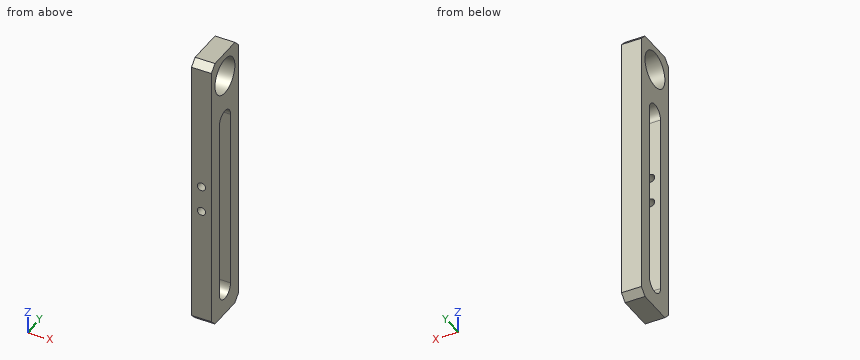
```python
from build123d import *

# Parameters (mm, degrees)
SKETCH1_W              = 85
SKETCH1_H              = 15
EXTRUDE1_DEPTH         = 6
M12X1_0_TAPPED_HOLE1_D = 11
CHAMFER1_SIZE          = 2
M3_TAPPED_HOLE1_D      = 2.5
M3_TAPPED_HOLE1_DEPTH  = 8.5
M3_TAPPED_HOLE1_TIP    = 0.751075774


with BuildPart() as part:
    # Sketch1 → Extrude1 (new body)
    with BuildSketch(Plane(origin=(0, 0, 0), x_dir=(0, 0, -1), z_dir=(1, 0, 0))):
        with Locations((42.5, -7.5)):
            Rectangle(SKETCH1_W, SKETCH1_H)
        with BuildLine():
            Line((22, -4.4), (77, -4.4))
            ThreePointArc((77, -4.4), (80.1, -7.5), (77, -10.6))
            Line((77, -10.6), (22, -10.6))
            ThreePointArc((22, -10.6), (18.9, -7.5), (22, -4.4))
        make_face(mode=Mode.SUBTRACT)
    extrude(amount=EXTRUDE1_DEPTH)

    # M12x1.0 Tapped Hole1 (through all)
    with Locations(Plane(origin=(6, 0, 0), x_dir=(0, 0, -1), z_dir=(1, 0, 0))):
        with Locations((7.5, -7.5)):
            Hole(M12X1_0_TAPPED_HOLE1_D / 2)

    # Chamfer1
    chamfer1_edges = [part.edges().sort_by_distance(p)[0] for p in [
        (3, 0, 0),
        (3, 0, -85),
        (3, -15, -85),
        (3, -15, 0),
    ]]
    chamfer(chamfer1_edges, length=CHAMFER1_SIZE)

    # M3 Tapped Hole1
    with Locations(Plane.XZ.offset(15)):
        with Locations((3, -40), (3, -48)):
            Hole(M3_TAPPED_HOLE1_D / 2, depth=M3_TAPPED_HOLE1_DEPTH)
            with Locations((0, 0, -(M3_TAPPED_HOLE1_DEPTH + M3_TAPPED_HOLE1_TIP / 2))):  # 118° drill point
                Cone(0, M3_TAPPED_HOLE1_D / 2, M3_TAPPED_HOLE1_TIP, mode=Mode.SUBTRACT)


solid = part.part
```
Verification items for the finished model (mm, model axes). Round coordinates to 2 decimals unless told otherwise and drop trailing zeros. Order: outer loops, then holes, each group sorted by start corner. A loop starts at its lowest first (then second) coordinate and runs counter-clockwise, first axis right, second up.
1) Material ranges on line 1 (Y direction, x = 2.8, z = -46.5); line 2 (Z direction, x = 2.2, y = -7.25); line 3 (Y direction, x = 3.45, z = -7.5), recorded low to high.
Geometry says:
line 1: y = -15 to -10.6, -4.4 to 0
line 2: z = -85 to -80.09, -18.91 to -12.99, -2.01 to 0
line 3: y = -15 to -13, -2 to 0
2) Cross-section at C-C, the plane z = -7.5. Record the cut outline in (x, y), plus the area to 3 significant figures.
Geometry says:
outline: (0, -15) - (6, -15) - (6, -13) - (0, -13) - close; (0, -2) - (6, -2) - (6, 0) - (0, 0) - close
area: 24.0 mm2
3) Cross-section at A-A, the plane z = -48. Record the cut outline in (x, y).
Geometry says:
outline: (0, -15) - (1.75, -15) - (1.75, -10.6) - (0, -10.6) - close; (0, -4.4) - (6, -4.4) - (6, 0) - (0, 0) - close; (4.25, -15) - (6, -15) - (6, -10.6) - (4.25, -10.6) - close
4) Cross-section at B-B, the plane x = 3. Record the cut outline in (y, z).
Geometry says:
outline: (-15, -83) - (-13, -85) - (-2, -85) - (0, -83) - (0, -2) - (-2, 0) - (-13, 0) - (-15, -2) - (-15, -38.75) - (-10.6, -38.75) - (-10.6, -22) arc R3.1 cw to (-4.4, -22) - (-4.4, -77) arc R3.1 cw to (-10.6, -77) - (-10.6, -49.25) - (-15, -49.25) - close; (-15, -46.75) - (-10.6, -46.75) - (-10.6, -41.25) - (-15, -41.25) - close; hole circle Ø11 at (-7.5, -7.5)
5) Cross-section at D-D, the plane y = -2.75. Record the cut outline in (x, z).
Geometry says:
outline: (0, -85) - (6, -85) - (6, -10.27) - (0, -10.27) - close; (0, -4.73) - (6, -4.73) - (6, 0) - (0, 0) - close
